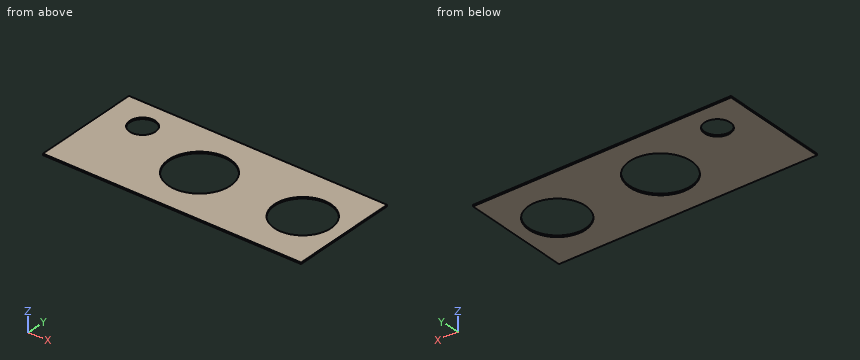
from build123d import *

# Parameters (mm, degrees)
SKETCH1_W           = 500
SKETCH1_H           = 210
BOSS_EXTRUDE1_DEPTH = 3
SKETCH2_R           = 55
SKETCH2_R_2         = 60
SKETCH2_R_3         = 25
CUT_EXTRUDE1_DEPTH  = 10


with BuildPart() as part:
    # Sketch1 → Boss-Extrude1 (new body)
    with BuildSketch(Plane.XY):
        with Locations((250, 105)):
            Rectangle(SKETCH1_W, SKETCH1_H)
    extrude(amount=BOSS_EXTRUDE1_DEPTH)

    # Sketch2 → Cut-Extrude1 (cut)
    with BuildSketch(Plane(origin=(492, 10, 3), x_dir=(1, 0, 0), z_dir=(0, 0, 1))):
        with Locations((-72, 95)):
            Circle(SKETCH2_R)
        with Locations((-272, 95)):
            Circle(SKETCH2_R_2)
        with Locations((-422, 145)):
            Circle(SKETCH2_R_3)
    extrude(amount=-CUT_EXTRUDE1_DEPTH, mode=Mode.SUBTRACT)


solid = part.part
Design review of the part built by this model. Coordinates are the model's own, in mm. Round coordinates to 2 decimals unless told otherwise and drop trailing zeros. Loops run counter-clockwise (first coordinate to the right, second up) from the corner with the lowest first, then second, coordinate; pieces in that order, holes last. Notation, with made-up numbers: (4, 85) - (12, 85) arc R9 ccw to (12, 99) - close; hole circle Ø5 at (-9.75, -30.75). An arc over 180 degrees is marked (long way). One line per item, written item: value. Start each with the question number.
1) Consider section C-C on z = 1.2. Give the boundary of the cut face in (x, y).
2) To check wall thickness, follow L1, parallel to Y at x = 218, z = 1.05; L2, parallel to X at y = 61.5, z = 1.6; L3, parallel to X at y = 101, z = 2.4. State the ranges of each line that lie inside material, in increasing order. Write a range as from..to.
3) Consider section A-A on y = 105. Give the boundary of the cut face in (x, z), then the cut area to 3 significant figures.
4) Consider section B-B on x = 420. Give the boundary of the cut face in (y, z).
5) Consider section D-D on y = 155. Give the boundary of the cut face in (x, z).
Reported:
1. outline: (0, 0) - (500, 0) - (500, 210) - (0, 210) - close; hole circle Ø50 at (70, 155); hole circle Ø120 at (220, 105); hole circle Ø110 at (420, 105)
2. L1: y = 0..45.03, 164.97..210
2. L2: x = 0..178.68, 261.32..386.34, 453.66..500
2. L3: x = 0..160.13, 279.87..365.15, 474.85..500
3. outline: (0, 0) - (160, 0) - (160, 3) - (0, 3) - close; (280, 0) - (365, 0) - (365, 3) - (280, 3) - close; (475, 0) - (500, 0) - (500, 3) - (475, 3) - close
3. area: 810 mm^2
4. outline: (0, 0) - (50, 0) - (50, 3) - (0, 3) - close; (160, 0) - (210, 0) - (210, 3) - (160, 3) - close
5. outline: (0, 0) - (45, 0) - (45, 3) - (0, 3) - close; (95, 0) - (186.83, 0) - (186.83, 3) - (95, 3) - close; (253.17, 0) - (397.09, 0) - (397.09, 3) - (253.17, 3) - close; (442.91, 0) - (500, 0) - (500, 3) - (442.91, 3) - close
